Check sheet for the modelled part. Datum: model origin and axes. Units: mm. Face numbers are marked on the shaded views. A direction names the side the tool comes from. Give positions to 0.01 mm unless a question says otherwise; leave off trailing zeros. Loops run counter-clockwise (first coordinate to the right, second up) from the corner with the lowest first, then second, coordinate; pieces in that order, holes last. Notation, with made-up numbers: (12.25, 60.25) -> (57.25, 60.25) arc R25 cw to (57.25, 75.25) -> close; hole circle Ø11 at (78, 77.25). An arc over 180 degrees is marked (long way). Write each question's results on one line, items separated by ' | '. Start each with the question number.
1. Tool access check on the marked faces 4 and 5. Record the directions out of +Z, -Z, +X, -X, +Y, -Y that give a thin tool (end or side, any length) a straight path to the whole face; none if there is none.
2. Mould release check, pull along X, two halves, no side actions. Record for the marked faces 1, 2 and 3: +X half, -X half, draft (parallel to the pull), parting line (faces both ways), or undercut.
3. Cross-section at C-C on y = -13. Record the boundary of the cut face in (x, z).
4. Gauge pin test, flat ends, axial feed: pin 1 Ø18 at (x, y) = (20, -55) entering from -Z; pin 2 Ø10 at (y, z) = (-52.5, 20.5) entering from -X; pin 3 Ø1 at (x, y) = (43.5, -23.5) entering from +Z; pin 4 Ø6 at (x, z) = (25, 23) entering from -Y. Record the tip position at first contact, or that the pin passes through.
5. Cross-section at D-D on x = 109. Record the boundary of the cut face in (y, z).
6. Cross-section at B-B on x = 20. Record the boundary of the cut face in (y, z).
7. Cross-section at A-A on z = 3. Record the boundary of the cut face in (x, y).
8. Material ranges on L1, parallel to Y at x = 15, z = 12; L2, parallel to X at y = -14, z = 12; L3, parallel to Z at x = -1.5, y = -63.5, recorded low to high. Write a range as from..to.
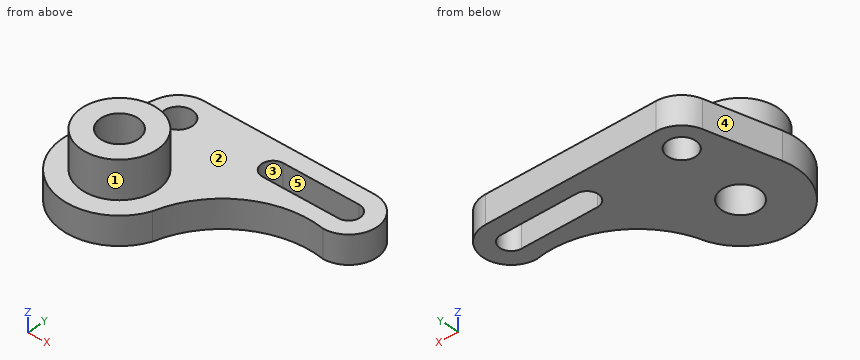
from build123d import *

# Parameters (mm, degrees)
LEVER_PLATE_DEPTH  = 15
HUB_PROFILE_R      = 20
HUB_40_DEPTH       = 20
HUB_BORE_PROFILE_R = 10
HUB_BORE_20_DEPTH  = 35
HOLE_PROFILE_R     = 7.5
HOLE_15_DEPTH      = 15
SLOT_12MM_DEPTH    = 15


with BuildPart() as part:
    # Lever Plate Profile → Lever Plate (new body)
    with BuildSketch(Plane.XY):
        with BuildLine():
            Line((15, 0), (105, 0))
            ThreePointArc((105, 0), (120, -15), (105, -30))
            ThreePointArc((105, -30), (69.260667374, -37.003214388), (47.752561519, -66.392775304))
            ThreePointArc((47.752561519, -66.392775304), (10.471129254, -83.44645184), (-9.015316087, -47.376914511))
            Line((-9.015316087, -47.376914511), (0.492341957, -11.188457255))
            ThreePointArc((0.492341957, -11.188457255), (5.83957264, -3.122013193), (15, 0))
        make_face()
    extrude(amount=LEVER_PLATE_DEPTH)

    # Hub Profile → Hub Ø40 (add)
    with BuildSketch(Plane.XY.offset(15)):
        with Locations((20, -55)):
            Circle(HUB_PROFILE_R)
    extrude(amount=HUB_40_DEPTH)

    # Hub Bore Profile → Hub Bore Ø20 (cut)
    with BuildSketch(Plane.XY.offset(35)):
        with Locations((20, -55)):
            Circle(HUB_BORE_PROFILE_R)
    extrude(amount=-HUB_BORE_20_DEPTH, mode=Mode.SUBTRACT)

    # Hole Profile → Hole Ø15 (cut)
    with BuildSketch(Plane.XY.offset(15)):
        with Locations((15, -15)):
            Circle(HOLE_PROFILE_R)
    extrude(amount=-HOLE_15_DEPTH, mode=Mode.SUBTRACT)

    # Slot Profile → Slot 12mm (cut)
    with BuildSketch(Plane.XY.offset(15)):
        with BuildLine():
            Line((65, -9), (105, -9))
            ThreePointArc((105, -9), (111, -15), (105, -21))
            Line((105, -21), (65, -21))
            ThreePointArc((65, -21), (59, -15), (65, -9))
        make_face()
    extrude(amount=-SLOT_12MM_DEPTH, mode=Mode.SUBTRACT)


solid = part.part
Geometry says:
1) face 4: +Z, -Z, -X, +Y | face 5: +Z, -Z
2) face 1: parting line | face 2: draft | face 3: undercut
3) outline: (0.02, 0) -> (7.77, 0) -> (7.77, 15) -> (0.02, 15) -> close; (22.23, 0) -> (59.34, 0) -> (59.34, 15) -> (22.23, 15) -> close; (110.66, 0) -> (119.87, 0) -> (119.87, 15) -> (110.66, 15) -> close
4) pin 1: through | pin 2: x = 0 | pin 3: z = 15 | pin 4: y = -74.9
5) outline: (-29.46, 0) -> (-19.47, 0) -> (-19.47, 15) -> (-29.46, 15) -> close; (-10.53, 0) -> (-0.54, 0) -> (-0.54, 15) -> (-10.53, 15) -> close
6) outline: (-85, 0) -> (-65, 0) -> (-65, 35) -> (-75, 35) -> (-75, 15) -> (-85, 15) -> close; (-45, 0) -> (-20.59, 0) -> (-20.59, 15) -> (-35, 15) -> (-35, 35) -> (-45, 35) -> close; (-9.41, 0) -> (0, 0) -> (0, 15) -> (-9.41, 15) -> close
7) outline: (-9.02, -47.38) arc R30 ccw to (47.75, -66.39) arc R50 cw to (105, -30) arc R15 ccw to (105, 0) -> (15, 0) arc R15 ccw to (0.49, -11.19) -> close; hole circle Ø15 at (15, -15); hole circle Ø20 at (20, -55); hole (65, -21) -> (105, -21) arc R6 ccw to (105, -9) -> (65, -9) arc R6 ccw to start
8) L1: -84.58..-63.66, -46.34..-22.5, -7.5..0 | L2: -0.25..7.57, 22.43..59.08, 110.92..119.97 | L3: 0..15
